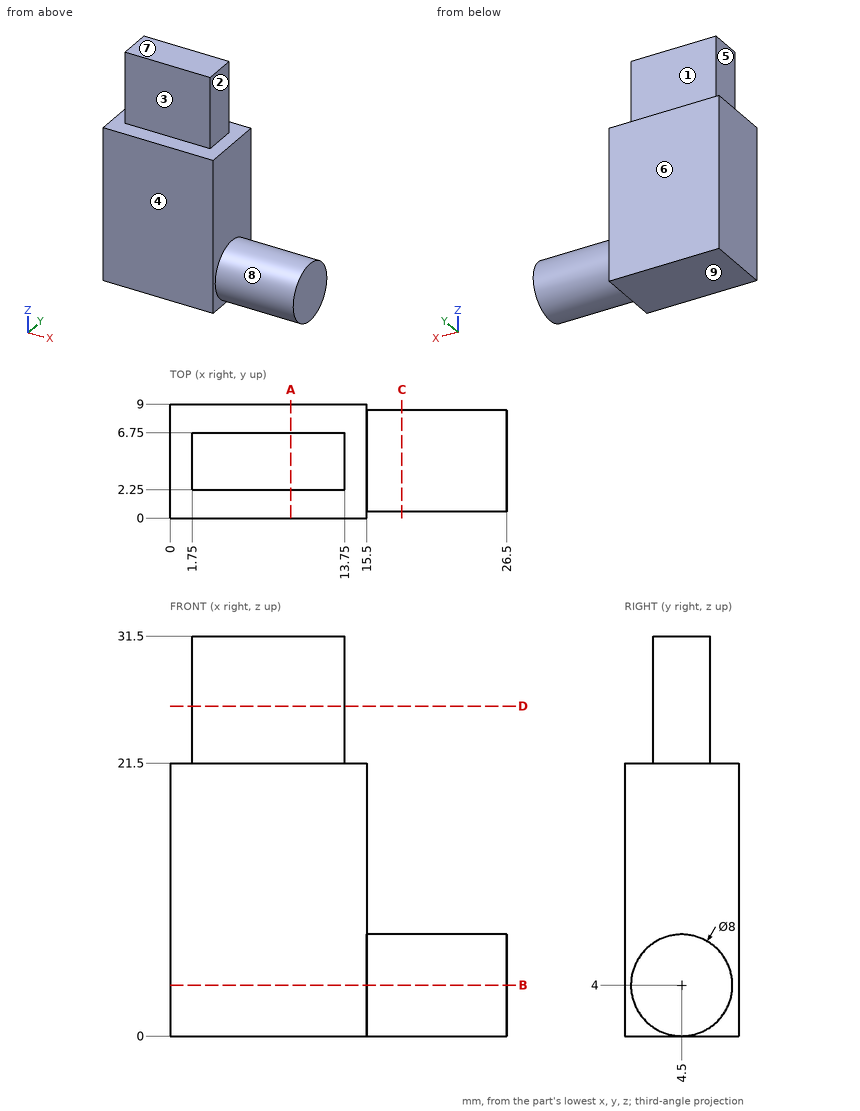
The drawing under review shows one solid part. Ordinate dimensions are in mm from its lowest x, y, z. A direction names the side the tool comes from. Coordinates: 2 decimals unless noted, no trailing zeros. Write each loop counter-clockwise with the first axis right and the second up, starting at its lowest first coordinate (ties: lowest second). Pieces come first, ordered by that corner, then holes. Notation, with made-up numbers: (76.5, 45) - (122.5, 45) arc R24 cw to (122.5, 76) - close; hole circle Ø8 at (6, -8). An arc over 180 degrees is marked (long way). Answer in a Markdown table with one row per item. Add a question column.
Q1. We need section B-B, the plane z = 4. State the section outline as (x, y) points, and give its area (4 significant figures).
Q2. For P1, Ø3, axis at y = 5.5, z = 19, coming from the +X side; P2, Ø1.5, axis at x = 14, z = 18.5, coming from the -Y side; P3, Ø1.5, axis at x = 6, z = 25.5, coming from the +Y side; P4, Ø3.5, axis at y = 4.5, z = 24.5, coming from the +X side, all flat-tipped, find the tip position at first contact; note any pin that passes through.
Q3. We need section C-C, the plane x = 18.25. State the section outline as (y, z) points, and give its area (3 significant figures).
Q4. Draft analysis for pull direction Z (two halves, no side actions). For the marked faces 6, 7, 8 and 9, state which applies: +Z half, -Z half, draft (parallel to the pull), parting line (faces both ways), or undercut.
Q5. We need section A-A, the plane x = 9.5. State the section outline as (y, z) points.
Q6. Tool access review of the marked faces 1, 2, 3, 4 and 5: name each direction out of +Z, -Z, +X, -X, +Y, -Y from which nothing blocks a thin tool from reaching the whole face with its end or side.
Q7. For probe 1 along Y at (x, z) = (13.25, 22); probe 2 along Z at (x, y) = (12.25, 7.25); probe 3 along X at (y, z) = (7, 16), list the stretches that pass through material, from the lowest coordinate up.
Q8. We need section D-D, the plane z = 26. State the section outline as (x, y) points, and give its area (3 significant figures).
Answer list:
| question | item | result |
|---|---|---|
| 1 | outline | (0, 0) - (15.5, 0) - (15.5, 0.5) - (26.5, 0.5) - (26.5, 8.5) - (15.5, 8.5) - (15.5, 9) - (0, 9) - close |
| 1 | area | 227.5 mm2 |
| 2 | P1 | stops at x = 15.5 |
| 2 | P2 | stops at y = 0 |
| 2 | P3 | stops at y = 6.75 |
| 2 | P4 | stops at x = 13.75 |
| 3 | outline | circle Ø8 at (4.5, 4) |
| 3 | area | 50.3 mm2 |
| 4 | face 6 | draft |
| 4 | face 7 | +Z half |
| 4 | face 8 | parting line |
| 4 | face 9 | -Z half |
| 5 | outline | (0, 0) - (9, 0) - (9, 21.5) - (6.75, 21.5) - (6.75, 31.5) - (2.25, 31.5) - (2.25, 21.5) - (0, 21.5) - close |
| 6 | face 1 | +Z, +X, -X, +Y |
| 6 | face 2 | +Z, +X, +Y, -Y |
| 6 | face 3 | +Z, +X, -X, -Y |
| 6 | face 4 | +Z, -Z, +X, -X, -Y |
| 6 | face 5 | +Z, -X, +Y, -Y |
| 7 | probe 1 | y = 2.25 to 6.75 |
| 7 | probe 2 | z = 0 to 21.5 |
| 7 | probe 3 | x = 0 to 15.5 |
| 8 | outline | (1.75, 2.25) - (13.75, 2.25) - (13.75, 6.75) - (1.75, 6.75) - close |
| 8 | area | 54.0 mm2 |
